from build123d import *

# Parameters (mm, degrees)
SKETCH1_W           = 16.7
SKETCH1_H           = 12
BOSS_EXTRUDE1_DEPTH = 2
SKETCH2_W           = 16.7
SKETCH2_H           = 2
BOSS_EXTRUDE2_DEPTH = 12
SKETCH4_W           = 2
SKETCH4_H           = 10
BOSS_EXTRUDE3_DEPTH = 16.7
M3_TAPPED_HOLE1_D   = 2.5
CUT_EXTRUDE1_DEPTH  = 1


with BuildPart() as part:
    # Sketch1 → Boss-Extrude1 (new body)
    with BuildSketch(Plane.XY):
        Rectangle(SKETCH1_W, SKETCH1_H)
    extrude(amount=BOSS_EXTRUDE1_DEPTH)

    # Sketch2 → Boss-Extrude2 (add)
    with BuildSketch(Plane.XY.offset(2)):
        with Locations((0, 7)):
            Rectangle(SKETCH2_W, SKETCH2_H)
        with Locations((0, -7)):
            Rectangle(SKETCH2_W, SKETCH2_H)
    extrude(amount=-BOSS_EXTRUDE2_DEPTH)

    # Sketch4 → Boss-Extrude3 (add)
    with BuildSketch(Plane.ZY.offset(8.35)):
        with Locations((-9, -13)):
            Rectangle(SKETCH4_W, SKETCH4_H)
        with Locations((-9, 13)):
            Rectangle(SKETCH4_W, SKETCH4_H)
    extrude(amount=-BOSS_EXTRUDE3_DEPTH)

    # M3 Tapped Hole1 (through all)
    with Locations(Plane.XY.offset(-8)):
        with Locations((0, -12.5), (0, 12.5)):
            Hole(M3_TAPPED_HOLE1_D / 2)

    # Sketch8 → Cut-Extrude1 (cut)
    with BuildSketch(Plane.ZY.offset(8.35)):
        Polygon((0, 6), (0, -6), (-10, -6), (-10, -18), (-8, -18), (-8, -8), (2, -8), (2, 8), (-8, 8), (-8, 18), (-10, 18), (-10, 6), align=None)
    extrude(amount=-CUT_EXTRUDE1_DEPTH, mode=Mode.SUBTRACT)


solid = part.part
The model under review builds one solid part; all positions refer to its coordinate system, in mm. A direction names the side the tool comes from. Round coordinates to 2 decimals unless told otherwise and drop trailing zeros. Order: outer loops, then holes, each group sorted by start corner. A loop starts at its lowest first (then second) coordinate and runs counter-clockwise, first axis right, second up. Notation, with made-up numbers: (-8, 49.5) -> (22, 49.5) arc R23 cw to (22, 76.5) -> close; hole circle Ø11 at (45.25, -22.75). An arc over 180 degrees is marked (long way). Return JSON: item names as keys, results as strings.
1. Take a section at B-B (x = 0). Write out the cut boundary in (y, z).
Answer block:
{"outline": "(-18, -10) -> (-13.75, -10) -> (-13.75, -8) -> (-18, -8) -> close; (-11.25, -10) -> (-6, -10) -> (-6, 0) -> (6, 0) -> (6, -10) -> (11.25, -10) -> (11.25, -8) -> (8, -8) -> (8, 2) -> (-8, 2) -> (-8, -8) -> (-11.25, -8) -> close; (13.75, -10) -> (18, -10) -> (18, -8) -> (13.75, -8) -> close"}
2. Insertion check: P1, Ø2, axis at x = 0, z = -3, coming from the +Y side; P2, Ø6, axis at x = 2.5, y = 2, coming from the -Z side; P3, Ø5, axis at x = 4, y = 13, coming from the +Z side. Each pin has a flat end and moves straight along its axis. Give the tip position at first contact, or say it passes through.
Answer block:
{"P1": "stops at y = 8", "P2": "stops at z = 0", "P3": "stops at z = -8"}
3. For L1, parallel to Y at x = 0, z = -9.05; L2, parallel to Y at x = 2, z = -0.25; L3, parallel to Y at x = -0.5, z = -8.25, list the stretches that pass through material, from the lowest coordinate up. Write a range as [from, to].
Answer block:
{"L1": "y = [-18, -13.75], [-11.25, -6], [6, 11.25], [13.75, 18]", "L2": "y = [-8, -6], [6, 8]", "L3": "y = [-18, -13.65], [-11.35, -6], [6, 11.35], [13.65, 18]"}
4. Take a section at C-C (y = -12.5). Write out the cut boundary in (x, z).
Answer block:
{"outline": "(-7.35, -10) -> (-1.25, -10) -> (-1.25, -8) -> (-7.35, -8) -> close; (1.25, -10) -> (8.35, -10) -> (8.35, -8) -> (1.25, -8) -> close"}
5. The part is to be moulded in two halves that separate along Y. For faces 1 (the face through (0, -11, -10)), 2 (the face through (0, 0, 0)), 3 (the face through (0, 18, -9)), say which applies: +Y half, -Y half, draft (parallel to the pull), parting line (faces both ways), or undercut.
Answer block:
{"face 1": "draft", "face 2": "undercut", "face 3": "+Y half"}
6. Take a section at D-D (x = 2.25). Write out the cut boundary in (y, z).
Answer block:
{"outline": "(-18, -10) -> (-6, -10) -> (-6, 0) -> (6, 0) -> (6, -10) -> (18, -10) -> (18, -8) -> (8, -8) -> (8, 2) -> (-8, 2) -> (-8, -8) -> (-18, -8) -> close"}
7. For faces 4 (the face through (0, -6, -5)), 5 (the face through (0.16, 13.74, -9.01)), 6 (the face through (0, -8, -3)), 7 (the face through (0, 8, -3)), list the 3-axis set-ups (+Z, -Z, +X, -X, +Y, -Y) from which the entire face can be reached by the end or side of a thin tool; tool diameter is ignored.
Answer block:
{"face 4": "-Z, +X, -X", "face 5": "+Z, -Z", "face 6": "+Z, +X, -X, -Y", "face 7": "+Z, +X, -X, +Y"}
8. Take a section at A-A (z = -6.5). Write out the cut boundary in (x, y), then the cut area to 3 significant figures.
Answer block:
{"outline": "(-7.35, -8) -> (8.35, -8) -> (8.35, -6) -> (-7.35, -6) -> close; (-7.35, 6) -> (8.35, 6) -> (8.35, 8) -> (-7.35, 8) -> close", "area": "62.8 mm²"}
